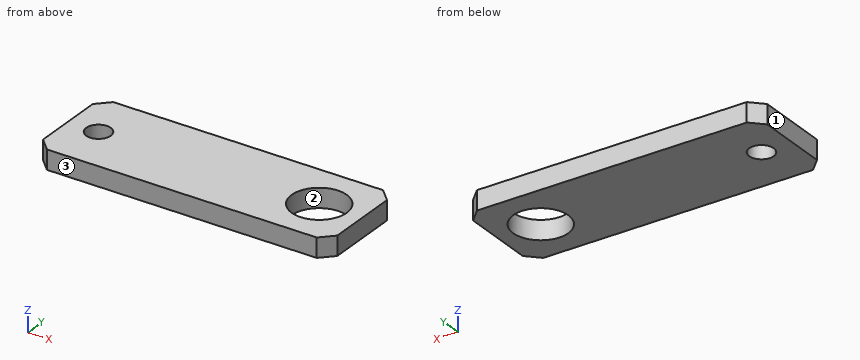
from build123d import *

# Parameters (mm, degrees)
SKETCH1_W      = 152.4
SKETCH1_H      = 50.8
SKETCH1_R      = 14.2875
SKETCH1_R_2    = 6.35
EXTRUDE1_DEPTH = 5
CHAMFER1_SIZE  = 6.35


with BuildPart() as part:
    # Sketch1 → Extrude1 (new, symmetric)
    with BuildSketch(Plane.XY):
        with Locations((3.175, 0)):
            Rectangle(SKETCH1_W, SKETCH1_H)
        with Locations((57.15, 0)):
            Circle(SKETCH1_R, mode=Mode.SUBTRACT)
        with Locations((-57.15, 0)):
            Circle(SKETCH1_R_2, mode=Mode.SUBTRACT)
    extrude(amount=EXTRUDE1_DEPTH, both=True)

    # Chamfer1
    chamfer1_edges = [part.edges().sort_by_distance(p)[0] for p in [
        (-73.025, 25.4, 0),
        (79.375, 25.4, 0),
        (79.375, -25.4, 0),
        (-73.025, -25.4, 0),
    ]]
    chamfer(chamfer1_edges, length=CHAMFER1_SIZE)


solid = part.part
Work out the finished part from the listing and answer in its coordinate system (mm). Face numbers are marked on the shaded views. Coordinates: 2 decimals unless noted, no trailing zeros. Order: outer loops, then holes, each group sorted by start corner. A loop starts at its lowest first (then second) coordinate and runs counter-clockwise, first axis right, second up. Notation, with made-up numbers: (36.5, 51) - (60.5, 51) arc R19 cw to (60.5, 64) - close; hole circle Ø8 at (-31, -31.5). An arc over 180 degrees is marked (long way). Put each result on its own line as item: value. Start each with the question number.
1) For a pull along Y with two mould halves and no side action, classify the marked faces 1, 2 and 3 as released by +Y, released by -Y, zero draft, split by the parting line, or undercut.
2) A flat-ended cylindrical pin translates along its axis: pin 1 (11.5 mm diameter, centred on x = -57.15, y = 0, fed in from +Z). Find the tip coordinate at first contact, or state that the pin passes through.
3) Find section D-D (x = 57.15). Give the vertices of the cut face in (y, z), plus the area to 3 significant figures.
4) Find the intervals of material crossed by line 1 (Y direction, x = 57.15, z = 2.5); line 2 (X direction, y = -1, z = -3.5) (3 decimals); line 3 (Y direction, x = -57.15, z = 2), in increasing order. Write a range as from..to.
5) Find section A-A (x = -57.15). Give the vertices of the cut face in (y, z), plus the area to 3 significant figures.
6) Find section C-C (z = 1.25). State how many separate pieces and enclosed holes the cut face has, plus the area to 3 significant figures.
7) Find section B-B (y = 0). Give the vertices of the cut face in (x, z) (1 decimal), plus the area to 3 significant figures.
Results list:
1. face 1: zero draft
1. face 2: undercut
1. face 3: released by -Y
2. pin 1: passes through
3. outline: (-25.4, -5) - (-14.29, -5) - (-14.29, 5) - (-25.4, 5) - close; (14.29, -5) - (25.4, -5) - (25.4, 5) - (14.29, 5) - close
3. area: 222 mm^2
4. line 1: y = -25.4..-14.29, 14.29..25.4
4. line 2: x = -73.025..-63.421, -50.879..42.898, 71.402..79.375
4. line 3: y = -25.4..-6.35, 6.35..25.4
5. outline: (-25.4, -5) - (-6.35, -5) - (-6.35, 5) - (-25.4, 5) - close; (6.35, -5) - (25.4, -5) - (25.4, 5) - (6.35, 5) - close
5. area: 381 mm^2
6. separate pieces: 1
6. enclosed holes: 2
6. area: 6,890 mm^2
7. outline: (-73, -5) - (-63.5, -5) - (-63.5, 5) - (-73, 5) - close; (-50.8, -5) - (42.9, -5) - (42.9, 5) - (-50.8, 5) - close; (71.4, -5) - (79.4, -5) - (79.4, 5) - (71.4, 5) - close
7. area: 1,110 mm^2
